Source: CAD feature listing. Evaluate the final solid. Frame: model axes, mm. A direction names the side the tool comes from. Coordinates: 2 decimals unless noted, no trailing zeros. Order: outer loops, then holes, each group sorted by start corner. A loop starts at its lowest first (then second) coordinate and runs counter-clockwise, first axis right, second up. Notation, with made-up numbers: (-10, 26) - (21, 26) arc R22 cw to (21, 44) - close; hole circle Ø4 at (-10, -19). An arc over 180 degrees is marked (long way). One line per question, with ' | ' between items. Start each with the question number.
(1) Line query: line 1 along X through (y, z) = (11.75, -55); line 2 along Z through (x, y) = (-58.5, 22); line 3 along Y through (x, z) = (-64, -129). Output: solid intervals per line, ascending.
(2) Contact query for flat-ended pins moving along their axis: P1, Ø24.5, axis at y = 45.5, z = -96.5, coming from the -X side; P2, Ø2, axis at x = -55.5, z = -91.5, coming from the +Y side; P3, Ø1, axis at x = -8.5, y = 30.5, coming from the +Z side. Output: stop coordinate, or through.
(3) Section D-D (x = -57). Return the cut outline in (y, z), then the cut area to 3 significant figures.
(4) Access query for faces 4 (the flat face through (-54, 30, -78)), 5 (the flat face through (-32, 90, -135)). Directions: +Z, -Z, +X, -X, +Y, -Y. A direction counts if a zero-diameter tool reaches every point of the face in a straight line with its end or side. Return the directions, or none.
(5) Section C-C (x = -21.5). Return the cut outline in (y, z).
(6) Section B-B (y = 62). Return the cut outline in (x, z), then the cut area to 3 significant figures.
(7) Section A-A (z = -47). Return the cut outline in (x, y).
(8) Draft query along X for faces 1 (the cylindrical face through (-71.37, 76.76, -134.79)), 2 (the flat face through (0, 36, -93)), 3 (the flat face through (-84, 20, -91)). Return one class per face: +X half, -X half, draft (parallel to the pull), parting line (faces both ways), or undercut.
from build123d import *

# Parameters (mm, degrees)
BRACKET_BODY_DEPTH     = 84
GUSSET_DEPTH           = 24
BASE_HOLES_SKETCH_R    = 10
BASE_HOLES_2X_20_DEPTH = 30
LUG_HOLE_SKETCH_R      = 10
LUG_HOLE_20_DEPTH      = 208
LUG_TOP_FILLET_R20_R   = 20


with BuildPart() as part:
    # Bracket Profile Sketch → Bracket Body (new body)
    with BuildSketch(Plane(origin=(0, 0, 0), x_dir=(0, 0, -1), z_dir=(1, 0, 0))):
        Polygon((0, 10), (0, 0), (150, 0), (150, 90), (120, 90), (120, 79.282032303), (120, 70), (120, 30), (34.641016151, 30), align=None)
    extrude(amount=-BRACKET_BODY_DEPTH)

    # Gusset Sketch → Gusset (add)
    with BuildSketch(Plane(origin=(0, 0, 0), x_dir=(0, 0, -1), z_dir=(1, 0, 0))):
        Polygon((34.641016151, 30), (120, 79.282032303), (120, 30), align=None)
    extrude(amount=-GUSSET_DEPTH)

    # Base Holes Sketch → Base Holes 2xØ20 (cut)
    with BuildSketch(Plane(origin=(0, 0, 0), x_dir=(1, 0, 0), z_dir=(0, 1, 0))):
        with Locations(Location((-64, 100, 0), (0, 0, 270))):
            Circle(BASE_HOLES_SKETCH_R)
        with Locations(Location((-64, 55, 0), (0, 0, 270))):
            Circle(BASE_HOLES_SKETCH_R)
    extrude(amount=BASE_HOLES_2X_20_DEPTH, mode=Mode.SUBTRACT)

    # Lug Hole Sketch → Lug Hole Ø20 (cut)
    with BuildSketch(Plane.XY):
        with Locations((-64, 70)):
            Circle(LUG_HOLE_SKETCH_R)
    extrude(amount=-LUG_HOLE_20_DEPTH, mode=Mode.SUBTRACT)

    # Lug Top Fillet R20
    lug_top_fillet_r20_edges = [part.edges().sort_by_distance(p)[0] for p in [
        (-84, 90, -135),
    ]]
    fillet(lug_top_fillet_r20_edges, radius=LUG_TOP_FILLET_R20_R)


solid = part.part
Response values:
1) line 1: x = -84 to -74, -54 to 0 | line 2: z = -150 to -108.35, -91.65 to -63.35, -46.65 to -20.78 | line 3: y = 0 to 60, 80 to 90
2) P1: stops at x = -24 | P2: stops at y = 30 | P3: stops at z = -34.64
3) outline: (0, -150) - (62.86, -150) - (62.86, -120) - (30, -120) - (30, -107.14) - (0, -107.14) - close; (0, -92.86) - (30, -92.86) - (30, -62.14) - (0, -62.14) - close; (0, -47.86) - (30, -47.86) - (30, -34.64) - (10, 0) - (0, 0) - close; (77.14, -150) - (90, -150) - (90, -120) - (77.14, -120) - close | area: 4,670 mm²
4) face 4: +Z, -X, +Y | face 5: +Z, -Z, +X, -X, +Y
5) outline: (0, -150) - (90, -150) - (90, -120) - (79.28, -120) - (10, 0) - (0, 0) - close
6) outline: (-84, -150) - (-70, -150) - (-70, -120) - (-84, -120) - close; (-58, -150) - (0, -150) - (0, -90.07) - (-24, -90.07) - (-24, -120) - (-58, -120) - close | area: 2,880 mm²
7) outline: (-84, 0) - (-70, 0) - (-70, 30) - (-84, 30) - close; (-58, 0) - (0, 0) - (0, 37.14) - (-24, 37.14) - (-24, 30) - (-58, 30) - close
8) face 1: undercut | face 2: +X half | face 3: -X half
